```python
from build123d import *

# Parameters (mm, degrees)
CHAMFER_1_SIZE      = 1
SKETCH_4_W          = 10
SKETCH_4_H          = 4.029490121
CUT_EXTRUDE_1_DEPTH = 69.000919111


with BuildPart() as part:
    # 草图1 → 旋转1 (revolve)
    with BuildSketch(Plane.XY, mode=Mode.PRIVATE) as revolve_1_sk:
        Polygon((0, 17.5), (0, 45.25), (18, 45.25), (18, 31.5), (23, 31.5), (23, 17.5), align=None)
    revolve(revolve_1_sk.sketch.rotate(Axis((0, 0, 0), (1, 0, 0)), 90), axis=Axis((0, 0, 0), (1, 0, 0)))

    # 草图2 → 切除-旋转1 (revolve, cut)
    with BuildSketch(Plane.XY, mode=Mode.PRIVATE) as cut_revolve_1_sk:
        Polygon((11.840143071, 33.8), (15.340759374, 45.25), (2.659240626, 45.25), (6.159856929, 33.8), align=None)
    revolve(cut_revolve_1_sk.sketch.rotate(Axis((0, 0, 0), (1, 0, 0)), 90), axis=Axis((0, 0, 0), (1, 0, 0)), mode=Mode.SUBTRACT)

    # 倒角1
    chamfer_1_edges = [part.edges().sort_by_distance(p)[0] for p in [
        (0, 0, -17.5),
        (23, 0, -17.5),
    ]]
    chamfer(chamfer_1_edges, length=CHAMFER_1_SIZE)

    # 草图4 → 切除-拉伸1 (cut, through all)
    with BuildSketch(Plane.ZY):
        with Locations((0, 18.785254892)):
            Rectangle(SKETCH_4_W, SKETCH_4_H)
    extrude(amount=-CUT_EXTRUDE_1_DEPTH, mode=Mode.SUBTRACT)


solid = part.part
```
Source: CAD feature listing. Evaluate the final solid. Frame: model axes, mm. A direction names the side the tool comes from. Give positions to 0.01 mm unless a question says otherwise; leave off trailing zeros. Write each loop counter-clockwise with the first axis right and the second up, starting at its lowest first coordinate (ties: lowest second). Pieces come first, ordered by that corner, then holes.
1. Section query D-D (x = 9.5). Return the cut outline in (y, z).
2. Pull-direction query (X, two-part tool) for faces 1 (the face through (23, 14, 14)), 2 (the face through (12.06, 33.7, -7.48)), 3 (the face through (1.35, -13.59, 43.16)); classes: +X half, -X half, draft (parallel to the pull), parting line (faces both ways), or undercut.
3. Section query A-A (z = 0). Return the cut outline in (x, y).
4. Section query C-C (x = 20). Return the cut outline in (y, z).
5. Access query for faces 4 (the face through (18, -31, 9)), 5 (the face through (0, -1, -19)), 6 (the face through (11, 20.8, 0)), 7 (the face through (0.84, -17.645, 0.709)), 8 (the face through (5.99, 20.91, -27.26)). Directions: +Z, -Z, +X, -X, +Y, -Y. A direction counts if a zero-diameter tool reaches every point of the face in a straight line with its end or side. Return the directions, or none.
6. First-contact query: pin 1 (1.5 mm diameter, centred on y = -34, z = -14, fed in from +X); pin 2 (3 mm diameter, centred on x = 8, y = 7, fed in from -Z); pin 3 (3 mm diameter, centred on x = 15.5, z = -2, fed in from -Y). Flat tips, straight axial feed; report the tip coordinate or a pass-through.
7. Section query B-B (y = 0). Return the cut outline in (x, z).
8. Material intervals for line 1 along Y through (x, z) = (17.5, 0); line 2 along Y through (x, z) = (7, 0); line 3 along X through (y, z) = (27.5, 35), sorted ascending.
Output values:
1. outline: circle Ø67.6 at (0, 0); hole (16.77, -5) - (20.8, -5) - (20.8, 5) - (16.77, 5) arc R17.5 ccw (long way) to start
2. face 1: +X half
2. face 2: undercut
2. face 3: draft
3. outline: (0, -45.25) - (2.66, -45.25) - (6.16, -33.8) - (11.84, -33.8) - (15.34, -45.25) - (18, -45.25) - (18, -31.5) - (23, -31.5) - (23, -18.5) - (22, -17.5) - (1, -17.5) - (0, -18.5) - close; (0, 20.8) - (23, 20.8) - (23, 31.5) - (18, 31.5) - (18, 45.25) - (15.34, 45.25) - (11.84, 33.8) - (6.16, 33.8) - (2.66, 45.25) - (0, 45.25) - close
4. outline: circle Ø63 at (0, 0); hole (16.77, -5) - (20.8, -5) - (20.8, 5) - (16.77, 5) arc R17.5 ccw (long way) to start
5. face 4: +X
5. face 5: +Z, -Z, -X, +Y, -Y
5. face 6: +X, -X
5. face 7: -X
5. face 8: none
6. pin 1: stops at x = 18
6. pin 2: stops at z = -33.35
6. pin 3: stops at y = -45.25
7. outline: (0, -45.25) - (2.66, -45.25) - (6.16, -33.8) - (11.84, -33.8) - (15.34, -45.25) - (18, -45.25) - (18, -31.5) - (23, -31.5) - (23, -18.5) - (22, -17.5) - (1, -17.5) - (0, -18.5) - close; (0, 18.5) - (1, 17.5) - (22, 17.5) - (23, 18.5) - (23, 31.5) - (18, 31.5) - (18, 45.25) - (15.34, 45.25) - (11.84, 33.8) - (6.16, 33.8) - (2.66, 45.25) - (0, 45.25) - close
8. line 1: y = -45.25 to -17.5, 20.8 to 45.25
8. line 2: y = -33.8 to -17.5, 20.8 to 33.8
8. line 3: x = 0 to 2.89, 15.11 to 18
